Part print with two shaded views. Sizes in mm from the minimum x, y, z corner. Round coordinates to 2 decimals unless told otherwise and drop trailing zeros. Order: outer loops, then holes, each group sorted by start corner. A loop starts at its lowest first (then second) coordinate and runs counter-clockwise, first axis right, second up. Notation, with made-up numbers: M 28,-34 L 65,-34 A23 cw 65,-19 Z; hole C 88.5,-21.75 d11. An arc over 180 degrees is marked long. Put each result on its own line as item: value.
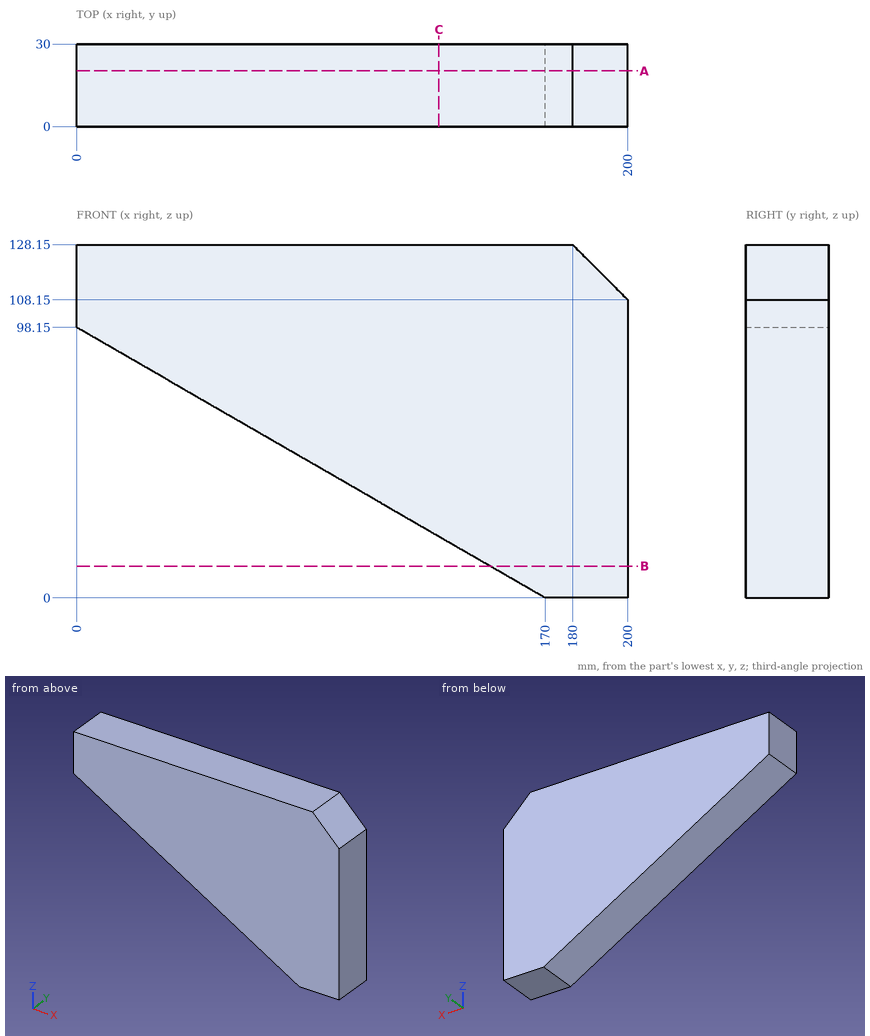
Item 1: Band-saw the part on B-B on z = 11.5. Give the cut face in (x, y), and give its area (3 significant figures).
Answers below:
outline: M 150.08,0 L 200,0 L 200,30 L 150.08,30 Z
area: 1,500 mm²
Item 2: Band-saw the part on A-A on y = 20.25. Give the cut face in (x, z), and give its area (3 significant figures).
Answers below:
outline: M 0,98.15 L 170,0 L 200,0 L 200,108.15 L 180,128.15 L 0,128.15 Z
area: 17,100 mm²
Item 3: Probe line 1 along Z through (x, y) = (86, 25.5); line 2 along Z through (x, y) = (83.5, 24.5); line 3 along X through (y, z) = (8.5, 51) (1 decimal). List the from-to ranges inside material, lowest first. Write a range as [from, to].
Answers below:
line 1: [48.5, 128.15]
line 2: [49.94, 128.15]
line 3: [81.7, 200]
Item 4: Band-saw the part on C-C on x = 131.5. Give the cut face in (y, z).
Answers below:
outline: M 0,22.23 L 30,22.23 L 30,128.15 L 0,128.15 Z
Item 5: Pin check, flat tips, straight feed: P1, Ø1, axis at y = 10, z = 97, coming from the -X side (1 decimal); P2, Ø5, axis at y = 8, z = 86, coming from the -X side (1 decimal); P3, Ø5, axis at x = 30.5, y = 11, coming from the -Z side. Stop position of each tip, or through.
Answers below:
P1: x = 1.1
P2: x = 16.7
P3: z = 79.1
